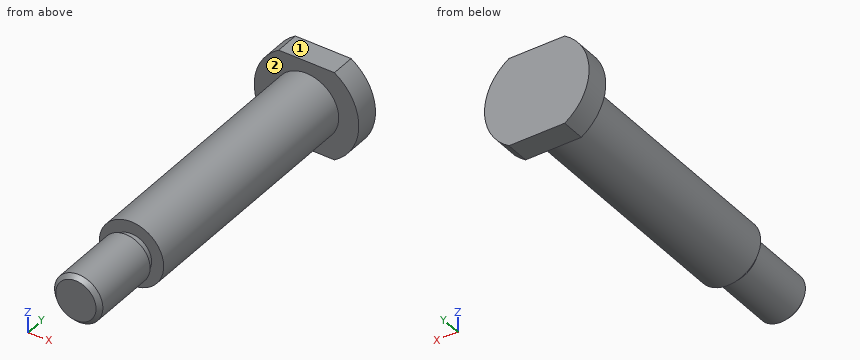
from build123d import *

# Parameters (mm, degrees)
SKETCH_1_R           = 4
EXTRUDE_1_DEPTH      = 31.5
SKETCH_2_R           = 3
EXTRUDE_2_DEPTH      = 10
SKETCH_3_R           = 6.5
EXTRUDE_3_DEPTH      = 3
SKETCH_4_OUTSIDE_W   = 24.63
SKETCH_4_OUTSIDE_H   = 24.63
SKETCH_4_OUTSIDE_W_2 = 13
SKETCH_4_OUTSIDE_H_2 = 11
CUT_EXTRUDE_1_DEPTH  = 46.439520244
CHAMFER_1_SIZE       = 0.5
SKETCH_5_W           = 0.5
SKETCH_5_H           = 1


with BuildPart() as part:
    # 草图1 → 凸台-拉伸1 (new body)
    with BuildSketch(Plane(origin=(0, 0, 0), x_dir=(1, 0, 0), z_dir=(0, 1, 0))):
        with Locations(Location((0, 0, 0), (0, 0, 270))):
            Circle(SKETCH_1_R)
    extrude(amount=EXTRUDE_1_DEPTH)

    # 草图2 → 凸台-拉伸2 (add)
    with BuildSketch(Plane.XZ):
        with Locations(Location((0, 0, 0), (0, 0, 270))):
            Circle(SKETCH_2_R)
    extrude(amount=EXTRUDE_2_DEPTH)

    # 草图3 → 凸台-拉伸3 (add)
    with BuildSketch(Plane(origin=(0, 31.5, 0), x_dir=(1, 0, 0), z_dir=(0, 1, 0))):
        with Locations(Location((0, 0, 0), (0, 0, 270))):
            Circle(SKETCH_3_R)
    extrude(amount=EXTRUDE_3_DEPTH)

    # 草图4 outside → 切除-拉伸1 (cut, through all)
    with BuildSketch(Plane(origin=(0, 34.5, 0), x_dir=(1, 0, 0), z_dir=(0, 1, 0))):
        Rectangle(SKETCH_4_OUTSIDE_W, SKETCH_4_OUTSIDE_H)
        Rectangle(SKETCH_4_OUTSIDE_W_2, SKETCH_4_OUTSIDE_H_2, mode=Mode.SUBTRACT)
    extrude(amount=-CUT_EXTRUDE_1_DEPTH, mode=Mode.SUBTRACT)

    # 倒角1
    chamfer_1_edges = [part.edges().sort_by_distance(p)[0] for p in [
        (0, -10, 3),
    ]]
    chamfer(chamfer_1_edges, length=CHAMFER_1_SIZE)

    # 草图5 → 切除-旋转1 (revolve, cut)
    with BuildSketch(Plane.XY, mode=Mode.PRIVATE) as cut_revolve_1_sk:
        with Locations((-2.75, -0.5)):
            Rectangle(SKETCH_5_W, SKETCH_5_H)
    revolve(cut_revolve_1_sk.sketch.rotate(Axis((0, 0, 0), (0, -1, 0)), 270), axis=Axis((0, 0, 0), (0, -1, 0)), mode=Mode.SUBTRACT)


solid = part.part
Input: part model. Units: mm. Frame: model coordinates. Face numbers are marked on the shaded views. A direction names the side the tool comes from. Give positions to 0.01 mm unless a question says otherwise; leave off trailing zeros. Loops run counter-clockwise (first coordinate to the right, second up) from the corner with the lowest first, then second, coordinate; pieces in that order, holes last. Notation, with made-up numbers: M 67.5,37 L 92.5,37 A9 ccw 92.5,47 Z; hole C 36,38.5 d1. An arc over 180 degrees is marked long. Use one line per item in the form item = value.
1. Section query D-D, the plane x = 5.5. Return the cut outline in (y, z).
Numbers:
outline = M 31.5,-3.46 L 34.5,-3.46 L 34.5,3.46 L 31.5,3.46 Z
2. Line query: L1, parallel to Z at x = 0.25, y = 13; L2, parallel to Y at x = -5.25, z = -1.75; L3, parallel to Y at x = -0.5, z = 3.5. Output: solid intervals per line, ascending.
Numbers:
L1 = -3.99 to 3.99
L2 = 31.5 to 34.5
L3 = 0 to 34.5
3. First-contact query: pin 1 (4 mm diameter, centred on x = -4.5, y = 12, fed in from +Z); pin 2 (3 mm diameter, centred on y = 25.5, z = -2, fed in from +X). Flat tips, straight axial feed; report the tip coordinate or a pass-through.
Numbers:
pin_1 = 3.12
pin_2 = 3.97
4. Section query C-C, the plane y = 13.5. Return the cut outline in (x, z), and give its area (3 significant figures).
Numbers:
outline = C 0,0 d8
area = 50.3 mm²
5. Section query A-A, the plane z = 0. Return the cut outline in (x, y).
Numbers:
outline = M -6.5,31.5 L -4,31.5 L -4,0 L -2.5,0 L -2.5,-1 L -3,-1 L -3,-9.5 L -2.5,-10 L 2.5,-10 L 3,-9.5 L 3,-1 L 2.5,-1 L 2.5,0 L 4,0 L 4,31.5 L 6.5,31.5 L 6.5,34.5 L -6.5,34.5 Z
6. Reachability of the marked faces 1 and 2 from +Z, -Z, +X, -X, +Y, -Y: full face, straight path, thin tool, end or side. Return the list, or none.
Numbers:
face_1 = +Z, +X, -X, +Y, -Y
face_2 = -Y
7. Section query B-B, the plane x = 0. Return the cut outline in (y, z), and give its area (3 significant figures).
Numbers:
outline = M -10,-2.5 L -9.5,-3 L -1,-3 L -1,-2.5 L 0,-2.5 L 0,-4 L 31.5,-4 L 31.5,-5.5 L 34.5,-5.5 L 34.5,5.5 L 31.5,5.5 L 31.5,4 L 0,4 L 0,2.5 L -1,2.5 L -1,3 L -9.5,3 L -10,2.5 Z
area = 344 mm²
